The figure shows three views and two pictorial views of one solid part (mm, origin at its lowest corner). Answer the questions. Coordinates: 2 decimals unless noted, no trailing zeros. Loops run counter-clockwise (first coordinate to the right, second up) from the corner with the lowest first, then second, coordinate; pieces in that order, holes last.
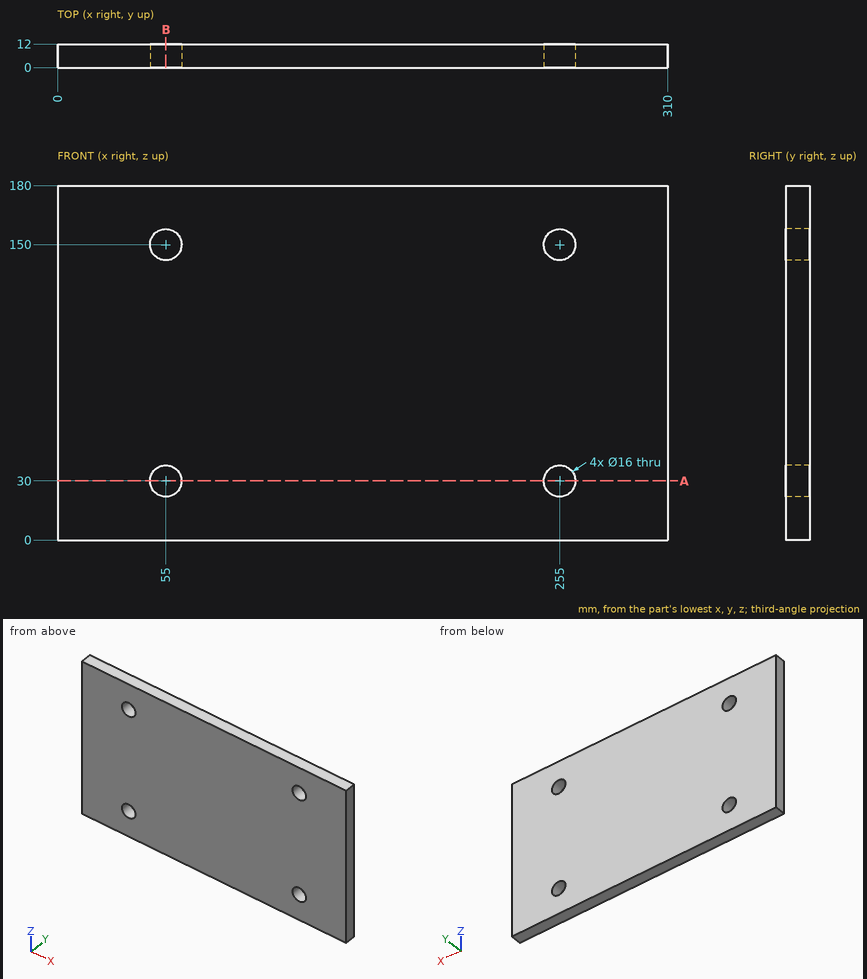
Q1. Straight lines are drawn through the part: probe 1 along X at (y, z) = (9.5, 150); probe 2 along X at (y, z) = (3.75, 31.5). For each, find the intervals that lie inside material, in ascending order.
Findings below:
probe 1: x = 0 to 47, 63 to 247, 263 to 310
probe 2: x = 0 to 47.14, 62.86 to 247.14, 262.86 to 310
Q2. A cutting plane is placed at A-A (z = 30). Give the vertices of the cut face in (x, y), then the cut area to 3 significant figures.
Findings below:
outline: (0, 0) - (47, 0) - (47, 12) - (0, 12) - close; (63, 0) - (247, 0) - (247, 12) - (63, 12) - close; (263, 0) - (310, 0) - (310, 12) - (263, 12) - close
area: 3,340 mm2
Q3. A flat-ended cylindrical pin translates along its axis: pin 1 Ø14.5 at (x, z) = (255, 30) entering from +Y. Find the tip coordinate at first contact, or state that the pin passes through.
Findings below:
pin 1: passes through
Q4. A cutting plane is placed at B-B (x = 55). Give the vertices of the cut face in (y, z), then the cut area to 3 significant figures.
Findings below:
outline: (0, 0) - (12, 0) - (12, 22) - (0, 22) - close; (0, 38) - (12, 38) - (12, 142) - (0, 142) - close; (0, 158) - (12, 158) - (12, 180) - (0, 180) - close
area: 1,780 mm2
